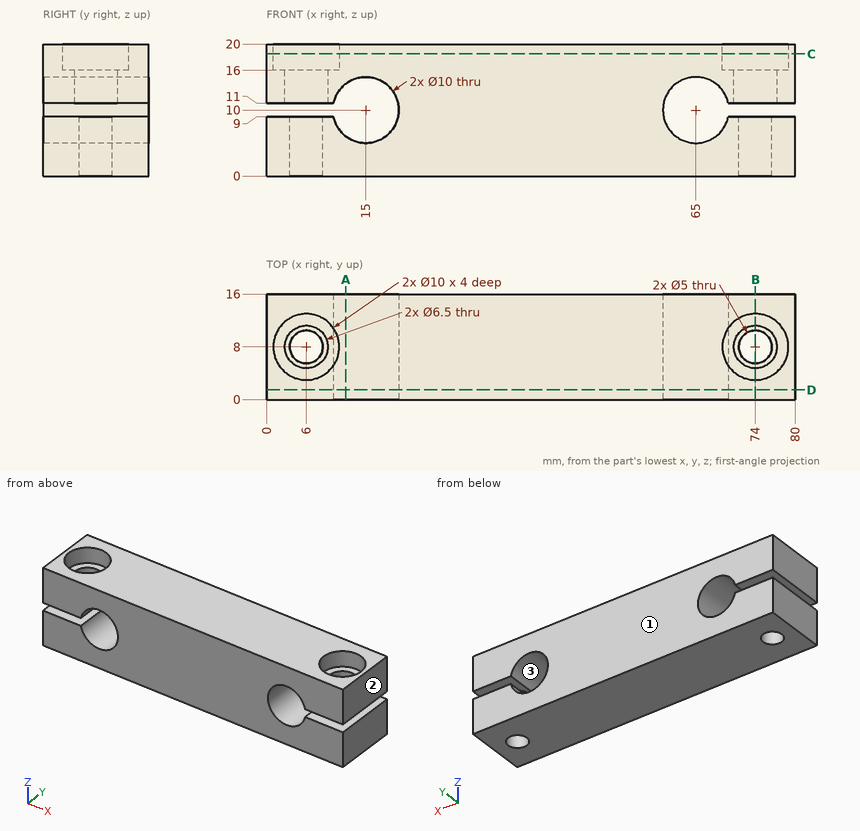
Geometry: see drawing. Coordinates: mm, zero at the bounding-box minimum. Give positions to 0.01 mm unless a question says otherwise; leave off trailing zeros. Loops run counter-clockwise (first coordinate to the right, second up) from the corner with the lowest first, then second, coordinate; pieces in that order, holes last. Notation, with made-up numbers: (68.5, 7) - (90.5, 7) arc R38 ccw to (90.5, 46) - close; hole circle Ø2 at (61.25, 79.25). An arc over 180 degrees is marked (long way). Use CSV: the item, a comma, the result in double quotes. Start each with the question number.
1. Draft query along X for the marked faces 1, 2 and 3. Return one class per face: +X half, -X half, draft (parallel to the pull), parting line (faces both ways), or undercut.
2. Section A-A (x = 12). Output: boundary loops of the cut face in (y, z).
3. Ray query, L1, parallel to X at y = 8, z = 3; L2, parallel to Z at x = 65, y = 12.5; L3, parallel to X at y = 8, z = 6.5. Return the intervals inside material, ascending.
4. Section C-C (z = 18.5). Output: boundary loops of the cut face in (x, y).
5. Section D-D (y = 1.5). Output: boundary loops of the cut face in (x, z), then the cut area to 3 significant figures.
6. Section B-B (x = 74). Output: boundary loops of the cut face in (y, z).
7. Pin query (flat end, axial travel): pin 1 (7.5 mm diameter, centred on x = 74, y = 8, fed in from +Z); pin 2 (6 mm diameter, centred on x = 6, y = 8, fed in from +Z). Return the tip coordinate at first contact, or that it passes through.
Response:
1,face 1,"draft"
1,face 2,"+X half"
1,face 3,"undercut"
2,outline,"(0, 0) - (16, 0) - (16, 6) - (0, 6) - close; (0, 14) - (16, 14) - (16, 20) - (0, 20) - close"
3,L1,"0 to 3.5, 8.5 to 71.5, 76.5 to 80"
3,L2,"0 to 5, 15 to 20"
3,L3,"0 to 3.5, 8.5 to 11.43, 18.57 to 61.43, 68.57 to 71.5, 76.5 to 80"
4,outline,"(0, 0) - (80, 0) - (80, 16) - (0, 16) - close; hole circle Ø10 at (6, 8); hole circle Ø10 at (74, 8)"
5,outline,"(0, 0) - (80, 0) - (80, 9) - (69.9, 9) arc R5 cw (long way) to (69.9, 11) - (80, 11) - (80, 20) - (0, 20) - (0, 11) - (10.1, 11) arc R5 cw (long way) to (10.1, 9) - (0, 9) - close"
5,area,"1,400 mm²"
6,outline,"(0, 0) - (5.5, 0) - (5.5, 9) - (0, 9) - close; (0, 11) - (4.75, 11) - (4.75, 16) - (3, 16) - (3, 20) - (0, 20) - close; (10.5, 0) - (16, 0) - (16, 9) - (10.5, 9) - close; (11.25, 11) - (16, 11) - (16, 20) - (13, 20) - (13, 16) - (11.25, 16) - close"
7,pin 1,"z = 16"
7,pin 2,"z = 9"
